Build history of the part. All positions in model axes, mm. A direction names the side the tool comes from. Round coordinates to 2 decimals unless told otherwise and drop trailing zeros. Loops run counter-clockwise (first coordinate to the right, second up) from the corner with the lowest first, then second, coordinate; pieces in that order, holes last. Notation, with made-up numbers: (-16, 47.25) - (13, 47.25) arc R32 ccw to (13, 83.25) - close; hole circle Ø7 at (77, -31.5). An arc over 180 degrees is marked (long way). One line per question, with ' | ' between items. Start each with the question number.
from build123d import *

# Parameters (mm, degrees)
EXTRUDE_1_DEPTH     = 100
CUT_EXTRUDE_1_DEPTH = 10


with BuildPart() as part:
    # Sketch 1 → Extrude 1 (new body)
    with BuildSketch(Plane.XY):
        Polygon((0, 0), (30, 0), (30, -3), (3, -3), (3, -30), (0, -30), align=None)
    extrude(amount=EXTRUDE_1_DEPTH)

    # Sketch 2 → Cut-Extrude 1 (cut)
    with BuildSketch(Plane(origin=(0, 0, 0), x_dir=(1, 0, 0), z_dir=(0, 1, 0))):
        with BuildLine():
            ThreePointArc((20, -50), (18.535533906, -46.464466094), (15, -45))
            Line((15, -45), (15, -55))
            ThreePointArc((15, -55), (18.535533906, -53.535533906), (20, -50))
        make_face()
        with BuildLine():
            Line((15, -55), (15, -45))
            ThreePointArc((15, -45), (10, -50), (15, -55))
        make_face()
    extrude(amount=-CUT_EXTRUDE_1_DEPTH, mode=Mode.SUBTRACT)


solid = part.part
1) Saw through at C-C on y = -14. Write the cut outline in (x, z), and give its area (3 significant figures).
2) Wall check: line 1 (Y direction, x = 28.25, z = 33); line 2 (X direction, y = -11.5, z = 35.5). Give the ranges that are in metal, low to high. Write a range as [from, to].
3) Tool access for faces 1 (the flat face through (0, -15, 49)), 2 (the flat face through (3, -16, 49)): list every direction of +Z, -Z, +X, -X, +Y, -Y with a clear straight run to the whole face (end or side of a thin tool).
4) Saw through at A-A on x = 13. Write the cut outline in (y, z), and give its area (3 significant figures).
5) Saw through at B-B on z = 34.5. Write the cut outline in (x, y).
6) Drop flat-ended pins along their axis: pin 1 (10 mm diameter, centred on x = 9.5, z = 23.5, fed in from -Y); pin 2 (8 mm diameter, centred on y = -16.5, z = 62, fed in from +X). Give the stop position or say it passes through.
7) Saw through at D-D on x = 27.75. Write the cut outline in (y, z), and give its area (3 significant figures).
Answer key:
1) outline: (0, 0) - (3, 0) - (3, 100) - (0, 100) - close | area: 300 mm²
2) line 1: [-3, 0] | line 2: [0, 3]
3) face 1: +Z, -Z, -X, +Y, -Y | face 2: +Z, -Z, +X, -Y
4) outline: (-3, 0) - (0, 0) - (0, 45.42) - (-3, 45.42) - close; (-3, 54.58) - (0, 54.58) - (0, 100) - (-3, 100) - close | area: 273 mm²
5) outline: (0, -30) - (3, -30) - (3, -3) - (30, -3) - (30, 0) - (0, 0) - close
6) pin 1: y = -3 | pin 2: x = 3
7) outline: (-3, 0) - (0, 0) - (0, 100) - (-3, 100) - close | area: 300 mm²
